Here's the drawing with two shaded views (mm, measured from the low corner). I have some questions. A direction names the side the tool comes from. Coordinates: 2 decimals unless noted, no trailing zeros. Write each loop counter-clockwise with the first axis right and the second up, starting at its lowest first coordinate (ties: lowest second). Pieces come first, ordered by that corner, then holes. Notation, with made-up numbers: (86.5, 31) -> (91.5, 31) arc R28 ccw to (91.5, 64) -> close; hole circle Ø3 at (14.5, 37). An arc over 180 degrees is marked (long way). Answer in a Markdown table with one row per item. Add a question column.
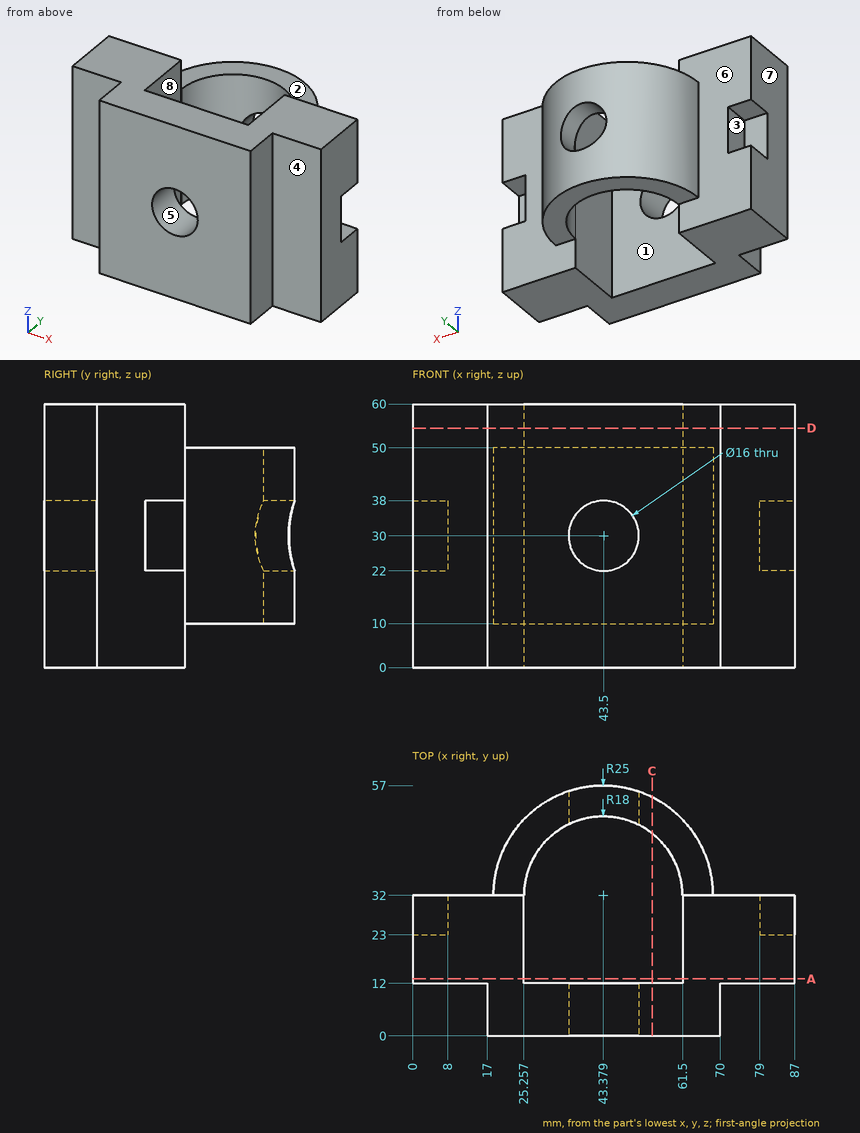
Q1. Imagine slicing it at C-C on x = 54.5. Please give me the cut outline in (y, z).
Q2. Imagine slicing it at D-D on z = 54.5. Please give me the cut outline in (x, y).
Q3. If we mould it in two halves opening along X, with no side actions, what happens to the marked faces 5, 6, 7 and 8? For each: pulls with the +X half, pulls with the -X half, needs draft (parallel to the pull), parting line crosses it, or undercut.
Q4. Imagine slicing it at A-A on y = 13. Please give me the cut outline in (x, z), plus the area to 4 significant figures.
Q5. I'm going to push flat-ended pins straight in: P1, Ø18.5, axis at x = 81.5, z = 28.5, coming from the -Y side; P2, Ø1.5, axis at x = 27, z = 37, coming from the +Y side; P3, Ø9.5, axis at y = 7, z = 28.5, coming from the +X side. Where does each tip first touch, or does it pass through?
Q6. I need wall thicknesses on line 1 (Z direction, x = 43.5, y = 51); line 2 (X direction, y = 31.5, z = 6.5); line 3 (Z direction, x = 43, y = 7) (1 decimal). Which ranges of each line are inside material? Lowest first, please. Write a range as [from, to].
Q7. For the marked faces 1, 2, 3 and 4, which set-ups out of +Z, -Z, +X, -X, +Y, -Y let a thin tool reach every point of the face, with its end or its side?
Result sheet:
| question | item | result |
|---|---|---|
| 1 | outline | (0, 0) -> (12, 0) -> (12, 60) -> (0, 60) -> close; (46.15, 10) -> (54.39, 10) -> (54.39, 50) -> (46.15, 50) -> close |
| 2 | outline | (0, 12) -> (17, 12) -> (17, 0) -> (70, 0) -> (70, 12) -> (87, 12) -> (87, 32) -> (61.5, 32) -> (61.51, 12) -> (25.26, 12) -> (25.26, 32) -> (0, 32) -> close |
| 3 | face 5 | undercut |
| 3 | face 6 | needs draft |
| 3 | face 7 | pulls with the -X half |
| 3 | face 8 | undercut |
| 4 | outline | (0, 0) -> (25.26, 0) -> (25.26, 60) -> (0, 60) -> close; (61.51, 0) -> (87, 0) -> (87, 60) -> (61.51, 60) -> close |
| 4 | area | 3,045 mm^2 |
| 5 | P1 | stops at y = 12 |
| 5 | P2 | stops at y = 51.51 |
| 5 | P3 | stops at x = 70 |
| 6 | line 1 | z = [10, 22], [38, 50] |
| 6 | line 2 | x = [0, 25.26], [61.5, 87] |
| 6 | line 3 | z = [0, 22], [38, 60] |
| 7 | face 1 | +Z, -Z |
| 7 | face 2 | +Z, +X, -X, +Y |
| 7 | face 3 | -X, +Y |
| 7 | face 4 | +Z, -Z, +X, -Y |
